Part model, mm, in its own coordinate system. A direction names the side the tool comes from. Give positions to 0.01 mm unless a question says otherwise; leave off trailing zeros. Write each loop counter-clockwise with the first axis right and the second up, starting at its lowest first coordinate (ties: lowest second). Pieces come first, ordered by that corner, then holes. Notation, with made-up numbers: (-15, -9) - (39, -9) arc R23 cw to (39, 3) - close; hole circle Ø9 at (50.5, 4). An arc over 180 degrees is marked (long way). Answer as a JSON object with one key per item and string values. Group by question number.
```python
from build123d import *

# Parameters (mm, degrees)
EXTRUDE_1_DEPTH     = 40.5
SKETCH_6_R          = 4.2
CUT_EXTRUDE_1_DEPTH = 20


with BuildPart() as part:
    # 草图1 → 凸台-拉伸1 (new body)
    with BuildSketch(Plane.XY):
        Polygon((-14.849242405, 9.192388155), (-10.394469683, 4.737615434), (-14.5, 0.632085117), (-14.5, -12.370057685), (-12.370057685, -14.5), (12.370057685, -14.5), (14.5, -12.370057685), (14.5, 12.370057685), (12.370057685, 14.5), (-0.632085117, 14.5), (-4.737615434, 10.394469683), (-9.192388155, 14.849242405), (-10.88944443, 13.15218613), (-10.182337649, 12.445079349), (-9.369164851, 13.258252147), (-7.247844507, 11.136931804), (-11.136931804, 7.247844507), (-13.258252147, 9.369164851), (-12.445079349, 10.182337649), (-13.15218613, 10.88944443), align=None)
    extrude(amount=-EXTRUDE_1_DEPTH)

    # 草图2 → 切除-旋转1 (revolve, cut)
    with BuildSketch(Plane(origin=(0, 0, 0), x_dir=(1, 0, 0), z_dir=(0, 1, 0)), mode=Mode.PRIVATE) as cut_revolve_1_sk:
        Polygon((8.5, 10), (8.5, 12.065), (14.065, 12.065), (15, 13), (15, 10), align=None)
    revolve(cut_revolve_1_sk.sketch.rotate(Axis((15, 0, -10), (-1, 0, 0)), 180), axis=Axis((15, 0, -10), (-1, 0, 0)), mode=Mode.SUBTRACT)

    # 草图3 → 切除-旋转2 (revolve, cut)
    with BuildSketch(Plane(origin=(0, 0, 0), x_dir=(1, 0, 0), z_dir=(0, 1, 0)), mode=Mode.PRIVATE) as cut_revolve_2_sk:
        Polygon((8.5, 35), (8.5, 37.065), (14.065, 37.065), (15, 38), (15, 35), align=None)
    revolve(cut_revolve_2_sk.sketch.rotate(Axis((15, 0, -35), (-1, 0, 0)), 180), axis=Axis((15, 0, -35), (-1, 0, 0)), mode=Mode.SUBTRACT)

    # 草图4 → 切除-旋转3 (revolve, cut)
    with BuildSketch(Plane(origin=(0, 0, 0), x_dir=(-0.7071067811865475, -0.7071067811865477, 0), z_dir=(0.7071067811865477, -0.7071067811865475, 0)), mode=Mode.PRIVATE) as cut_revolve_3_sk:
        Polygon((-14, -0.5), (-16.5, -0.5), (-15.62, 0.38), (-15.62, 40.12), (-16.5, 41), (-14, 41), align=None)
    revolve(cut_revolve_3_sk.sketch.rotate(Axis((9.899494937, 9.899494937, -41), (0, 0, 1)), 315), axis=Axis((9.899494937, 9.899494937, -41), (0, 0, 1)), mode=Mode.SUBTRACT)

    # 草图5 → 切除-旋转4 (revolve, cut)
    with BuildSketch(Plane(origin=(0, 0, 0), x_dir=(-0.7071067811865475, -0.7071067811865477, 0), z_dir=(0.7071067811865477, -0.7071067811865475, 0)), mode=Mode.PRIVATE) as cut_revolve_4_sk:
        Polygon((14, -0.5), (11.5, -0.5), (12.38, 0.38), (12.38, 40.12), (11.5, 41), (14, 41), align=None)
    revolve(cut_revolve_4_sk.sketch.rotate(Axis((-9.899494937, -9.899494937, -41), (0, 0, 1)), 315), axis=Axis((-9.899494937, -9.899494937, -41), (0, 0, 1)), mode=Mode.SUBTRACT)

    # 草图6 → 切除-拉伸1 (cut)
    with BuildSketch(Plane.XY):
        Circle(SKETCH_6_R)
    extrude(amount=-CUT_EXTRUDE_1_DEPTH, mode=Mode.SUBTRACT)


solid = part.part
```
1) Drill centre lines: line 1 along Y through (x, z) = (9.85, -35) (3 decimals); line 2 along Y through (x, z) = (0, -4); line 3 along Y through (x, z) = (9.25, -4). Where is each one in solid material? Low to high. Write a range as from..to.
2) Saw through at D-D (z = -35). List the corners of the cut face in (x, y) (1 decimal).
3) Drop flat-ended pins along their axis: P1, Ø11, axis at x = 0, y = 0, coming from the +Z side; P2, Ø4, axis at x = 0.5, y = 1, coming from the +Z side; P3, Ø4, axis at y = -3, z = -25, coming from the -X side; P4, Ø2, axis at y = -0.5, z = -34, coming from the +X side. Give the stop position or say it passes through.
4) Saw through at B-B (y = 0). List the corners of the cut face in (x, z) (3 decimals).
5) Which spindle directions (+Z, -Z, +X, -X, +Y, -Y) get a long thin tool onto all of the face, cutting with end or side? Do faces 5 (the cylindrical face through (11.321, 0.091, -12.063)), 6 (the flat face through (6, 14.5, -20)), 7 (the flat face through (-10.03, 14.01, -19.97)), 8 (the flat face through (-12.653, 6.996, -19.966)). Say none if no direction does.
6) Saw through at A-A (z = -10). State how many separate pieces and enclosed holes the cut face has, and give its area (3 significant figures).
7) Saw through at C-C (x = 0). List the corners of the cut face in (y, z), and give its area (3 significant figures).
8) Two-plate mould, pull along X, no slides. Class faces 1 (the cylindrical face through (11.445, 10.386, -20.528)), 2 (the flat face through (8.5, 0, -35)), 3 (the flat face through (-14.5, -6, -20)), 4 (the flat face through (3, 4, 0)): +X half, -X half, draft (parallel to the pull), parting line (faces both ways), or undercut.
Checks:
{
 "1": {"line 1": "-14.5..-2.065, 2.065..8.28, 11.519..14.5", "line 2": "-14.5..-4.2, 4.2..14.5", "line 3": "-14.5..8.42, 11.38..14.5"},
 "2": {"outline": "(-14.8, 9.2) - (-10.4, 4.7) - (-14.5, 0.6) - (-14.5, -12.4) - (-12.4, -14.5) - (12.4, -14.5) - (14.5, -12.4) - (14.5, -2.5) - (14.1, -2.1) - (8.5, -2.1) - (8.5, 2.1) - (14.1, 2.1) - (14.5, 2.5) - (14.5, 12.4) - (12.4, 14.5) - (-0.6, 14.5) - (-4.7, 10.4) - (-9.2, 14.8) - (-10.9, 13.2) - (-10.2, 12.4) - (-9.4, 13.3) - (-7.2, 11.1) - (-11.1, 7.2) - (-13.3, 9.4) - (-12.4, 10.2) - (-13.2, 10.9) - close; hole circle Ø3.2 at (-9.9, -9.9); hole circle Ø3.2 at (9.9, 9.9)"},
 "3": {"P1": "z = 0", "P2": "z = -20", "P3": "x = -14.5", "P4": "x = 14.12"},
 "4": {"outline": "(-14.5, -40.5) - (14.5, -40.5) - (14.5, -37.5) - (14.065, -37.065) - (8.5, -37.065) - (8.5, -32.935) - (14.065, -32.935) - (14.5, -32.5) - (14.5, -12.5) - (14.065, -12.065) - (8.5, -12.065) - (8.5, -7.935) - (14.065, -7.935) - (14.5, -7.5) - (14.5, 0) - (4.2, 0) - (4.2, -20) - (-4.2, -20) - (-4.2, 0) - (-14.5, 0) - close"},
 "5": {"face 5": "+X", "face 6": "+Z, -Z, +X, +Y", "face 7": "+Z, -Z, -X, +Y", "face 8": "+Z, -Z, -X"},
 "6": {"separate pieces": "1", "enclosed holes": "3", "area": "672 mm2"},
 "7": {"outline": "(-14.5, -40.5) - (14.5, -40.5) - (14.5, 0) - (4.2, 0) - (4.2, -20) - (-4.2, -20) - (-4.2, 0) - (-14.5, 0) - close", "area": "1,010 mm2"},
 "8": {"face 1": "undercut", "face 2": "+X half", "face 3": "-X half", "face 4": "draft"}
}
